from build123d import *

# Parameters (mm, degrees)
SKETCH1_R           = 3
BOSS_EXTRUDE1_DEPTH = 30
SKETCH2_W           = 30
SKETCH2_H           = 24
SKETCH2_H_2         = 6
CUT_EXTRUDE1_DEPTH  = 30
CUT_EXTRUDE2_DEPTH  = 10
SKETCH4_W           = 29.142135624
SKETCH4_H           = 18
CUT_EXTRUDE3_DEPTH  = 12


with BuildPart() as part:
    # Sketch1 → Boss-Extrude1 (new body)
    with BuildSketch(Plane.XY):
        with BuildLine():
            Line((1.925621669, 9.059337681), (3.188348425, 15))
            Line((3.188348425, 15), (49.261728674, 15))
            ThreePointArc((49.261728674, 15), (56.761728674, 7.5), (49.261728674, 0))
            Line((49.261728674, 0), (9.261728674, 0))
            ThreePointArc((9.261728674, 0), (3.433133963, 2.780097067), (1.925621669, 9.059337681))
        make_face()
        with Locations((9.261728674, 7.5)):
            Circle(SKETCH1_R, mode=Mode.SUBTRACT)
        with Locations((49.261728674, 7.5)):
            Circle(SKETCH1_R, mode=Mode.SUBTRACT)
    extrude(amount=BOSS_EXTRUDE1_DEPTH)

    # Sketch2 → Cut-Extrude1 (cut)
    with BuildSketch(Plane(origin=(0, 15, 0), x_dir=(1, 0, 0), z_dir=(0, 1, 0))):
        with Locations((1.761728674, -15)):
            Rectangle(SKETCH2_W, SKETCH2_H)
        with Locations((56.761728674, 0)):
            Rectangle(SKETCH2_W, SKETCH2_H_2)
        with Locations((56.761728674, -30)):
            Rectangle(SKETCH2_W, SKETCH2_H_2)
    extrude(amount=-CUT_EXTRUDE1_DEPTH, mode=Mode.SUBTRACT)

    # Sketch3 → Cut-Extrude2 (cut)
    with BuildSketch(Plane(origin=(0, 15, 0), x_dir=(1, 0, 0), z_dir=(0, 1, 0))):
        Polygon((-3.238271326, -3), (36.761728674, -3), (36.761728674, -6), (65.37522755, -6), (65.37522755, -24), (36.761728674, -24), (36.761728674, -27), (-3.238271326, -27), align=None)
    extrude(amount=-CUT_EXTRUDE2_DEPTH, mode=Mode.SUBTRACT)

    # Sketch4 → Cut-Extrude3 (cut)
    with BuildSketch(Plane(origin=(0, 5, 0), x_dir=(1, 0, 0), z_dir=(0, 1, 0))):
        with Locations((56.332796486, -15)):
            Rectangle(SKETCH4_W, SKETCH4_H)
    extrude(amount=-CUT_EXTRUDE3_DEPTH, mode=Mode.SUBTRACT)


solid = part.part
Model file for the job. Use its own axes, mm. A direction names the side the tool comes from. Coordinates: 2 decimals unless noted, no trailing zeros. Write each loop counter-clockwise with the first axis right and the second up, starting at its lowest first coordinate (ties: lowest second). Pieces come first, ordered by that corner, then holes. Notation, with made-up numbers: (38.25, 52) - (56.25, 52) arc R20 ccw to (56.25, 62) - close; hole circle Ø4 at (86, 48.5). An arc over 180 degrees is marked (long way). Write each question's results on one line, items separated by ' | '. Start each with the question number.
1) Probe line 1 along Z through (x, y) = (20, 5.25); line 2 along Z through (x, y) = (43, 3.5); line 3 along X through (y, z) = (7.5, 0.9). List the from-to ranges inside material, lowest first. Write a range as from..to.
2) Cut at B-B (x = 16). Write the cut outline in (y, z), then the cut area to 3 significant figures.
3) Cut at C-C (z = 25.25). Write the cut outline in (x, y), then the cut area to 3 significant figures.
4) Flat gauge pins, fed straight in: P1, Ø1.5, axis at y = 9.5, z = 1.5, coming from the +X side; P2, Ø0.9, axis at y = 11, z = 25, coming from the -X side; P3, Ø6, axis at x = 12, z = 22.5, coming from the -Y side; P4, Ø5, axis at x = 49, y = 9, coming from the -Z side. Where does each tip first touch, or does it go through?
5) Cut at D-D (y = 11.5). Write the cut outline in (x, z), then the cut area to 3 significant figures.
6) 3-axis set-ups, long thin cutter, end or side, ignore diameter. For faces 1 (the face through (41.762, 8, 2)), 2 (the face through (46, 8, 27)), 3 (the face through (46.6, 9.3, 24)): which of +Z, -Z, +X, -X, +Y, -Y reach the whole face in a straight line?
7) Mould opens along Y. For faces 4 (the face through (41.762, 8, 29)), 5 (the face through (26, 15, 28)), 6 (the face through (46.265, 7.632, 25.479)) say: pulls with the +Y half, pulls with the -Y half, needs draft (parallel to the pull), parting line crosses it, or undercut.
8) Cut at A-A (y = 7.5). Count the separate pieces of the cut face and the enclosed holes in it, then the cut area to 3 significant figures.
Returned:
1) line 1: 0..3, 27..30 | line 2: 3..6, 24..27 | line 3: 1.76..6.26, 12.26..41.76
2) outline: (0, 0) - (15, 0) - (15, 3) - (0, 3) - close; (0, 27) - (15, 27) - (15, 30) - (0, 30) - close | area: 90.0 mm^2
3) outline: (16.76, 0) - (49.26, 0) arc R7.5 ccw to (49.26, 15) - (36.76, 15) - (36.76, 5) - (16.76, 5) - close; hole circle Ø6 at (49.26, 7.5) | area: 348 mm^2
4) P1: x = 41.76 | P2: x = 36.76 | P3: through | P4: z = 3
5) outline: (2.44, 0) - (41.76, 0) - (41.76, 3) - (55.61, 3) - (55.61, 6) - (36.76, 6) - (36.76, 3) - (2.44, 3) - close; (2.44, 27) - (36.76, 27) - (36.76, 24) - (55.61, 24) - (55.61, 27) - (41.76, 27) - (41.76, 30) - (2.44, 30) - close | area: 349 mm^2
6) face 1: -Z, +X, +Y, -Y | face 2: +Z, +X, +Y, -Y | face 3: +X, +Y
7) face 4: needs draft | face 5: pulls with the +Y half | face 6: undercut
8) separate pieces: 6 | enclosed holes: 0 | area: 288 mm^2
